```python
from build123d import *

# Parameters (mm, degrees)
M42X1_5_TAPPED_HOLE1_D     = 40.5
M42X1_5_TAPPED_HOLE1_DEPTH = 88.5
M42X1_5_TAPPED_HOLE1_TIP   = 12.167427535


with BuildPart() as part:
    # Sketch1 → Revolve1 (revolve)
    with BuildSketch(Plane.XY, mode=Mode.PRIVATE) as revolve1_sk:
        Polygon((20, 0), (40, 0), (40, 30), (37.5, 30), (27.5, 25), (24, 25), (20, 21), align=None)
    revolve(revolve1_sk.sketch.rotate(Axis((0, 0, 0), (0, 1, 0)), 90), axis=Axis((0, 0, 0), (0, 1, 0)))

    # M42X1.5 Tapped Hole1
    with Locations(Plane(origin=(0, 0, 0), x_dir=(-1, 0, 0), z_dir=(0, -1, 0))):
        with Locations((0, 0)):
            Hole(M42X1_5_TAPPED_HOLE1_D / 2, depth=M42X1_5_TAPPED_HOLE1_DEPTH)
            with Locations((0, 0, -(M42X1_5_TAPPED_HOLE1_DEPTH + M42X1_5_TAPPED_HOLE1_TIP / 2))):  # 118° drill point
                Cone(0, M42X1_5_TAPPED_HOLE1_D / 2, M42X1_5_TAPPED_HOLE1_TIP, mode=Mode.SUBTRACT)


solid = part.part
```
The listing builds one solid part. Answer for the finished solid, in the listing's coordinates (mm). A direction names the side the tool comes from. Coordinates: 2 decimals unless noted, no trailing zeros. Write each loop counter-clockwise with the first axis right and the second up, starting at its lowest first coordinate (ties: lowest second). Pieces come first, ordered by that corner, then holes. Notation, with made-up numbers: (-30.5, 86.25) - (1.5, 86.25) arc R13 cw to (1.5, 104.25) - close; hole circle Ø8 at (63, 7). An arc over 180 degrees is marked (long way). One line per item, written item: value.
1) Consider line 1 along Y through (x, z) = (-7, -25.5); line 2 along X through (y, z) = (18, 17.5); line 3 along Z through (x, y) = (-18.5, 3.5). Determine where each line is inside the solid, lowest interval first. Write a range as from..to.
Geometry check:
line 1: y = 0..25
line 2: x = -35.97..-10.19, 10.19..35.97
line 3: z = -35.46..-8.23, 8.23..35.46
2) A tool of negligible diameter and unlimited length cuts with its end or side. For faces 4 (the flat face through (-23, 25, 8)), 5 (the flat face through (-36, 30, -12)), from which of +Z, -Z, +X, -X, +Y, -Y can it reach the whole face along a straight path? Write none if from no direction.
Geometry check:
face 4: +Y
face 5: +Z, -Z, +X, -X, +Y
3) Each of these flat-tipped pins is pushed along its axis until it touches: pin 1 Ø3 at (x, y) = (8, 23) entering from +Z; pin 2 Ø6 at (x, y) = (-8, 22.5) entering from +Z; pin 3 Ø2 at (x, y) = (31.5, 17.5) entering from +Z. Where does it stop, or does it pass through?
Geometry check:
pin 1: stops at z = 39.47
pin 2: stops at z = 39.69
pin 3: stops at z = 25.88
4) Find section C-C (y = 4). Give the vertices of the cut face in (x, z), and give its area (3 significant figures).
Geometry check:
outline: circle Ø80 at (0, 0); hole circle Ø40.5 at (0, 0)
area: 3,740 mm2
5) Find section B-B (x = 0). Give the vertices of the cut face in (y, z), and give its area (3 significant figures).
Geometry check:
outline: (0, -40) - (30, -40) - (30, -37.5) - (25, -27.5) - (25, -24) - (21.25, -20.25) - (0, -20.25) - close; (0, 20.25) - (21.25, 20.25) - (25, 24) - (25, 27.5) - (30, 37.5) - (30, 40) - (0, 40) - close
area: 1,050 mm2
6) For a pull along X with two mould halves and no side action, classify faces 1 (the conical face through (-6.137, 21.432, -19.489)), 2 (the cylindrical face through (-1.76, 15.21, 39.96)), 3 (the flat face through (-9.4, 0, -18.3)) as pulls with the +X half, pulls with the -X half, needs draft (parallel to the pull), parting line crosses it, or undercut.
Geometry check:
face 1: undercut
face 2: parting line crosses it
face 3: needs draft
7) Find section A-A (z = 0). Give the vertices of the cut face in (x, y).
Geometry check:
outline: (-40, 0) - (-20.25, 0) - (-20.25, 21.25) - (-24, 25) - (-27.5, 25) - (-37.5, 30) - (-40, 30) - close; (20.25, 0) - (40, 0) - (40, 30) - (37.5, 30) - (27.5, 25) - (24, 25) - (20.25, 21.25) - close
